For this review, take the finished solid that the model builds, in its own axes (mm). Face numbers are marked on the shaded views. A direction names the side the tool comes from. Give positions to 0.01 mm unless a question says otherwise; leave off trailing zeros. Order: outer loops, then holes, each group sorted by start corner. A loop starts at its lowest first (then second) coordinate and runs counter-clockwise, first axis right, second up.
from build123d import *

# Parameters (mm, degrees)
HUB_PROFILE_20_R        = 10
SHAFT_HUB_20X71_DEPTH   = 71
KEYED_BORE_10_REACH     = 74.395
ROCKER_START            = -48
ROCKER_ARM_DEPTH        = 18
ARM_FILLET_R3_R         = 3
SADDLE_BLOCK_DEPTH      = 2
SADDLE_BLOCK_DEPTH_BACK = 8
CONNECTING_WEB_DEPTH    = 6
FORK_SLOT_DEPTH         = 90.549416149
FORK_SLOT_DEPTH_BACK    = 90.549416149


with BuildPart() as part:
    # Hub Profile Ø20 → Shaft Hub Ø20x71 (new body)
    with BuildSketch(Plane(origin=(0, 0, 0), x_dir=(0, 0, -1), z_dir=(1, 0, 0))):
        Circle(HUB_PROFILE_20_R)
    extrude(amount=SHAFT_HUB_20X71_DEPTH)

    # Keyed Bore Profile → Keyed Bore Ø10 (cut, up to next)
    with BuildSketch(Plane(origin=(71, 0, 0), x_dir=(0, 0, -1), z_dir=(1, 0, 0)), mode=Mode.PRIVATE) as keyed_bore_10_sk1:
        with BuildLine():
            Line((-2, -4.582575695), (-2, -7.5))
            Line((-2, -7.5), (2, -7.5))
            Line((2, -7.5), (2, -4.582575695))
            ThreePointArc((2, -4.582575695), (0, 5), (-2, -4.582575695))
        make_face()
    keyed_bore_10_tool1 = extrude(keyed_bore_10_sk1.sketch, amount=-KEYED_BORE_10_REACH, mode=Mode.PRIVATE) & part.part
    add(keyed_bore_10_tool1.solids().sort_by_distance((71, -0.731497, 0))[0], mode=Mode.SUBTRACT)

    # Rocker Arm Profile → Rocker Arm (add)
    with BuildSketch(Plane(origin=(71, 0, 0), x_dir=(0, 0, -1), z_dir=(1, 0, 0)).offset(ROCKER_START)):
        with BuildLine():
            Line((-10, 0), (-10, 16))
            Line((-10, 16), (10, 16))
            Line((10, 16), (10, 0))
            ThreePointArc((10, 0), (0, 10), (-10, 0))
        make_face()
    extrude(amount=ROCKER_ARM_DEPTH)

    # Arm Fillet R3
    arm_fillet_r3_edges = [part.edges().sort_by_distance(p)[0] for p in [
        (23, 16, 0),
        (41, 16, 0),
    ]]
    fillet(arm_fillet_r3_edges, radius=ARM_FILLET_R3_R)



with BuildPart() as body_2:
    # Saddle Block Profile → Saddle Block (new, two sides: drawn at the far end of the back side and taken through both)
    with BuildSketch(Plane.ZY.offset(-SADDLE_BLOCK_DEPTH_BACK)):
        with BuildLine():
            Line((22, -33), (22, -46.228756555))
            ThreePointArc((22, -46.228756555), (13, -17), (4, -46.228756555))
            Line((4, -46.228756555), (4, -33))
            ThreePointArc((4, -33), (13, -24), (22, -33))
        make_face()
    extrude(amount=SADDLE_BLOCK_DEPTH + SADDLE_BLOCK_DEPTH_BACK)


with BuildPart() as part_1:
    add(part.part)

    add(body_2.part)  # Connecting Web merges body 2
    # Connecting Web Profile → Connecting Web (add)
    with BuildSketch(Plane.ZY):
        with BuildLine():
            ThreePointArc((-2.664036214, -36.261590024), (7.135607706, -18.113465715), (26.679934465, -24.701843999))
            Line((26.679934465, -24.701843999), (8.549959041, 5.186347501))
            ThreePointArc((8.549959041, 5.186347501), (9.63066951, 2.692620433), (10, 0))
            ThreePointArc((10, 0), (1.024639854, -9.947367148), (-9.790022634, -2.038493765))
            Line((-9.790022634, -2.038493765), (-2.664036214, -36.261590024))
        make_face()
    extrude(amount=-CONNECTING_WEB_DEPTH)

    # Fork Slot Profile → Fork Slot (cut, two sides: drawn at the far end of the back side and taken through both)
    with BuildSketch(Plane.XY.offset(-FORK_SLOT_DEPTH_BACK)):
        with BuildLine():
            Line((26, 16), (26, 11.01))
            ThreePointArc((26, 11.01), (32, 5.01), (38, 11.01))
            Line((38, 11.01), (38, 16))
            Line((38, 16), (26, 16))
        make_face()
    extrude(amount=FORK_SLOT_DEPTH + FORK_SLOT_DEPTH_BACK, mode=Mode.SUBTRACT)


solid = part_1.part
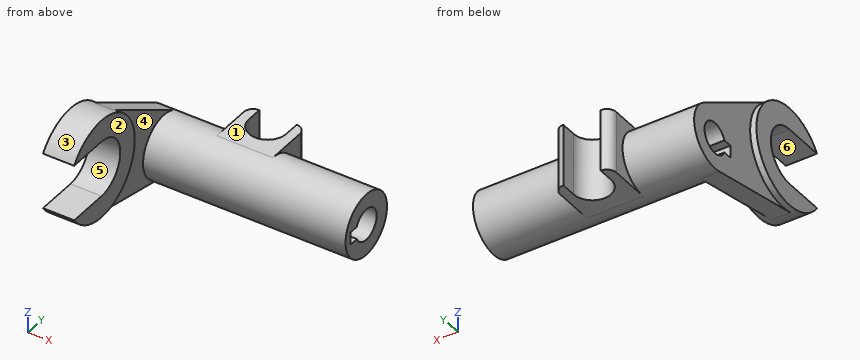
1) To check wall thickness, follow line 1 (Y direction, x = 42.5, z = 0); line 2 (X direction, y = -20.5, z = 1.5); line 3 (Z direction, x = 21, y = 0). State the ranges of each line that lie inside material, in increasing order.
Answer sheet:
line 1: y = -10 to -7.5, 5 to 10
line 2: x = 0 to 6
line 3: z = -10 to -5, 5 to 10
2) We need section D-D on z = 13. Give the boundary of the cut face in (x, y).
Answer sheet:
outline: (-2, -24) - (8, -24) - (8, -17) - (6, -17) - (6, -2.15) - (0, -2.15) - (0, -17) - (-2, -17) - close
3) Clearance check with flat-ended pins moving along their axes: pin 1 (9 mm diameter, centred on y = 0, z = 0, fed in from -X); pin 2 (0.9 mm diameter, centred on x = 51.5, y = -6.5, fed in from +Z); pin 3 (5 mm diameter, centred on x = 0.5, y = -42, fed in from +Z); pin 4 (17.5 mm diameter, centred on x = 34, y = 11.5, fed in from +Z). State where each tip first meets the part, or that it passes through.
Answer sheet:
pin 1: passes through
pin 2: stops at z = 7.96
pin 3: stops at z = 27.62
pin 4: stops at z = 10
4) We need section B-B on z = 0. Give the boundary of the cut face in (x, y), then the cut area to 3 significant figures.
Answer sheet:
outline: (-2, -42.33) - (8, -42.33) - (8, -23.67) - (6, -23.67) - (6, -10) - (71, -10) - (71, -7.5) - (0, -7.5) - (0, -23.67) - (-2, -23.67) - close; (0, 5) - (71, 5) - (71, 10) - (41, 10) - (41, 13) arc R3 ccw to (38, 16) - (38, 11.01) arc R6 cw to (26, 11.01) - (26, 16) arc R3 ccw to (23, 13) - (23, 10) - (0, 10) - close
area: 789 mm2
5) Draft analysis for pull direction Y (two halves, no side actions). For the marked faces 4, 5 and 6, state which applies: +Y half, -Y half, draft (parallel to the pull), parting line (faces both ways), or undercut.
Answer sheet:
face 4: undercut
face 5: -Y half
face 6: draft
6) Tool access review of the marked faces 1, 2 and 3: name each direction out of +Z, -Z, +X, -X, +Y, -Y from which nothing blocks a thin tool from reaching the whole face with its end or side.
Answer sheet:
face 1: +Z, +X, +Y, -Y
face 2: +Z, -Z, +X, -Y
face 3: none
7) We need section C-C on y = -38. Give the boundary of the cut face in (x, z).
Answer sheet:
outline: (-2, -2.2) - (8, -2.2) - (8, 4) - (-2, 4) - close; (-2, 22) - (8, 22) - (8, 28.2) - (-2, 28.2) - close
8) We need section A-A on x = 32. Give the boundary of the cut face in (y, z).
Answer sheet:
outline: (0, -10) - (5.01, -10) - (5.01, 10) - (0, 10) arc R10 ccw to start; hole (-7.5, -2) - (-4.58, -2) arc R5 ccw (long way) to (-4.58, 2) - (-7.5, 2) - close
